CAD build for the part. Positions are in the model's coordinates, mm. Face numbers are marked on the shaded views. A direction names the side the tool comes from. Round coordinates to 2 decimals unless told otherwise and drop trailing zeros. Loops run counter-clockwise (first coordinate to the right, second up) from the corner with the lowest first, then second, coordinate; pieces in that order, holes last.
```python
from build123d import *

# Parameters (mm, degrees)
SKETCH1_R           = 25
SKETCH1_R_2         = 19
BOSS_EXTRUDE1_DEPTH = 5
SKETCH2_R           = 10
BOSS_EXTRUDE2_DEPTH = 12
SKETCH3_R           = 19
SKETCH3_R_2         = 10
BOSS_EXTRUDE3_DEPTH = 2
CUT_EXTRUDE1_DEPTH  = 50


with BuildPart() as part:
    # Sketch1 → Boss-Extrude1 (new, symmetric)
    with BuildSketch(Plane(origin=(0, 0, 0), x_dir=(1, 0, 0), z_dir=(0, 1, 0))):
        with Locations(Location((0, 0, 0), (0, 0, 270))):
            Circle(SKETCH1_R)
        with Locations(Location((0, 0, 0), (0, 0, 270))):
            Circle(SKETCH1_R_2, mode=Mode.SUBTRACT)
    extrude(amount=BOSS_EXTRUDE1_DEPTH, both=True)



with BuildPart() as body_2:
    # Sketch2 → Boss-Extrude2 (new body)
    with BuildSketch(Plane(origin=(0, 5, 0), x_dir=(1, 0, 0), z_dir=(0, 1, 0))):
        with Locations(Location((0, 0, 0), (0, 0, 270))):
            Circle(SKETCH2_R)
    extrude(amount=-BOSS_EXTRUDE2_DEPTH)


with BuildPart() as part_1:
    add(part.part)

    add(body_2.part)  # Boss-Extrude3 merges body 2
    # Sketch3 → Boss-Extrude3 (add, symmetric)
    with BuildSketch(Plane(origin=(0, 0, 0), x_dir=(1, 0, 0), z_dir=(0, 1, 0))):
        with Locations(Location((0, 0, 0), (0, 0, 270))):
            Circle(SKETCH3_R)
        with Locations(Location((0, 0, 0), (0, 0, 270))):
            Circle(SKETCH3_R_2, mode=Mode.SUBTRACT)
    extrude(amount=BOSS_EXTRUDE3_DEPTH, both=True)

    # Sketch4 → Cut-Extrude1 (cut)
    with BuildSketch(Plane.XZ.offset(7)):
        Polygon((-4.242640687, 0), (0, 4.242640687), (4.242640687, 0), (0, -4.242640687), align=None)
    extrude(amount=-CUT_EXTRUDE1_DEPTH, mode=Mode.SUBTRACT)


solid = part_1.part
```
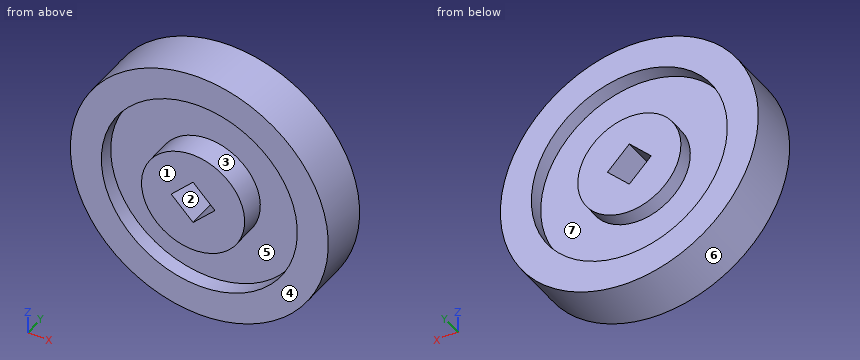
Item 1: Probe line 1 (Y direction, x = 22.5, z = -9); line 2 (Y direction, x = 3, z = -18.5); line 3 (Z direction, x = -15.5, y = -4). List the from-to ranges inside material, lowest first.
Answers follow:
line 1: y = -5 to 5
line 2: y = -2 to 2
line 3: z = -19.62 to -10.99, 10.99 to 19.62
Item 2: Two-plate mould, pull along Z, no slides. Class the marked faces 4, 5, 6 and 7: released by +Z, released by -Z, zero draft, split by the parting line, or undercut.
Answers follow:
face 4: zero draft
face 5: undercut
face 6: split by the parting line
face 7: undercut
Item 3: Flat gauge pins, fed straight in: P1, Ø1.5, axis at x = 13.5, z = 2, coming from the -Y side; P2, Ø2, axis at x = -5, y = 0.5, coming from the +Z side; P3, Ø3, axis at y = -0.5, z = -3, coming from the -X side. Where does each tip first touch, or does it go through?
Answers follow:
P1: stops at y = -2
P2: stops at z = 24.68
P3: stops at x = -24.95
Item 4: Cut at D-D, the plane x = 7. Give the cut face in (y, z).
Answers follow:
outline: (-7, -7.14) - (-2, -7.14) - (-2, -17.66) - (-5, -17.66) - (-5, -24) - (5, -24) - (5, -17.66) - (2, -17.66) - (2, -7.14) - (5, -7.14) - (5, 7.14) - (2, 7.14) - (2, 17.66) - (5, 17.66) - (5, 24) - (-5, 24) - (-5, 17.66) - (-2, 17.66) - (-2, 7.14) - (-7, 7.14) - close
Item 5: Cut at C-C, the plane z = -15.5. Give the cut face in (x, y).
Answers follow:
outline: (-19.62, -5) - (-10.99, -5) - (-10.99, -2) - (10.99, -2) - (10.99, -5) - (19.62, -5) - (19.62, 5) - (10.99, 5) - (10.99, 2) - (-10.99, 2) - (-10.99, 5) - (-19.62, 5) - close
Item 6: Cut at A-A, the plane y = -3.25. Give the cut face in (x, z).
Answers follow:
outline: circle Ø50 at (0, 0); circle Ø20 at (0, 0); hole circle Ø38 at (0, 0); hole (-4.24, 0) - (0, -4.24) - (4.24, 0) - (0, 4.24) - close
Item 7: Cut at B-B, the plane y = -6. Give the cut face in (x, z).
Answers follow:
outline: circle Ø20 at (0, 0); hole (-4.24, 0) - (0, -4.24) - (4.24, 0) - (0, 4.24) - close
Item 8: 3-axis set-ups, long thin cutter, end or side, ignore diameter. For the marked faces 1, 2 and 3: which of +Z, -Z, +X, -X, +Y, -Y reach the whole face in a straight line?
Answers follow:
face 1: +Z, -Z, +X, -X, -Y
face 2: +Y, -Y
face 3: -Y
